from build123d import *

# Parameters (mm, degrees)
SKETCH1_W           = 15
SKETCH1_H           = 20
BOSS_EXTRUDE1_DEPTH = 50
FILLET1_RADIUS      = 10
FILLET1_LENGTH      = 15
SKETCH2_R           = 4
CUT_EXTRUDE1_DEPTH  = 54.150729064
CUT_EXTRUDE2_DEPTH  = 54.150729064
FILLET2_R           = 5
SKETCH4_R           = 3.5
BOSS_EXTRUDE2_DEPTH = 6
DOME1_FACE_RADIUS   = 3.5
DOME1_HEIGHT        = 3
CUT_EXTRUDE3_DEPTH  = 55.371407941


with BuildPart() as part:
    # Sketch1 → Boss-Extrude1 (new body)
    with BuildSketch(Plane(origin=(0, 0, 0), x_dir=(1, 0, 0), z_dir=(0, 1, 0))):
        Rectangle(SKETCH1_W, SKETCH1_H)
    extrude(amount=BOSS_EXTRUDE1_DEPTH)

    # Fillet1: full round fillet: the end face becomes a half cylinder, R = half its width
    fillet1_face = Plane((0, 0, 0), x_dir=(-1, 0, 0), z_dir=(0, -1, 0))  # on the end face: x along it, z out of the body
    fillet1_slab = fillet1_face.offset(-FILLET1_RADIUS / 2) * Box(FILLET1_LENGTH, 2 * FILLET1_RADIUS, FILLET1_RADIUS, mode=Mode.PRIVATE)  # the body's end, R deep
    fillet1_round = Plane((0, 10, 0), x_dir=(0, -1, 0), z_dir=(-1, 0, 0)) * Cylinder(FILLET1_RADIUS, FILLET1_LENGTH, mode=Mode.PRIVATE)  # its axis R under the face
    add(fillet1_slab - fillet1_round, mode=Mode.SUBTRACT)

    # Sketch2 → Cut-Extrude1 (cut, through all)
    with BuildSketch(Plane.ZY.offset(7.5)):
        with Locations((0, 10)):
            Circle(SKETCH2_R)
    extrude(amount=-CUT_EXTRUDE1_DEPTH, mode=Mode.SUBTRACT)

    # Sketch3 → Cut-Extrude2 (cut, through all)
    with BuildSketch(Plane.ZY.offset(7.5)):
        with BuildLine():
            Line((0, 20), (0, 50))
            Line((0, 50), (10, 50))
            Line((10, 50), (10, 10))
            ThreePointArc((10, 10), (7.071067812, 17.071067812), (0, 20))
        make_face()
    extrude(amount=-CUT_EXTRUDE2_DEPTH, mode=Mode.SUBTRACT)

    # Fillet2
    fillet2_edges = [part.edges().sort_by_distance(p)[0] for p in [
        (0, 20, 0),
    ]]
    fillet(fillet2_edges, radius=FILLET2_R)

    # Sketch4 → Boss-Extrude2 (add)
    with BuildSketch(Plane.XY):
        with Locations(Location((0, 25, 0), (0, 0, 194.18798624))):
            Circle(SKETCH4_R)
    extrude(amount=BOSS_EXTRUDE2_DEPTH)

    # Dome1: a dome of height H over a round flat face of radius A is a cap of a sphere of radius (A * A + H * H) / (2 * H)
    dome1_r = (DOME1_FACE_RADIUS * DOME1_FACE_RADIUS + DOME1_HEIGHT * DOME1_HEIGHT) / (2 * DOME1_HEIGHT)
    dome1_base = Plane((0, 25, 6), z_dir=(0, 0, 1))
    with Locations(dome1_base.offset(DOME1_HEIGHT - dome1_r)):
        dome1_ball = Sphere(dome1_r, mode=Mode.PRIVATE)
    add(split(dome1_ball, bisect_by=dome1_base, keep=Keep.TOP, mode=Mode.PRIVATE))

    # Sketch5 → Cut-Extrude3 (cut, through all)
    with BuildSketch(Plane(origin=(0, 0, -10), x_dir=(-1, 0, 0), z_dir=(0, 0, -1))):
        with BuildLine():
            Line((3.05, 50), (3.05, 32.634868852))
            ThreePointArc((3.05, 32.634868852), (0, 29.584868852), (-3.05, 32.634868852))
            Line((-3.05, 32.634868852), (-3.05, 50))
            ThreePointArc((-3.05, 50), (0, 53.05), (3.05, 50))
        make_face()
    extrude(amount=-CUT_EXTRUDE3_DEPTH, mode=Mode.SUBTRACT)


solid = part.part
Can you work these out from the model? Positions are in its coordinate system, mm. A direction names the side the tool comes from. Give positions to 0.01 mm unless a question says otherwise; leave off trailing zeros. Loops run counter-clockwise (first coordinate to the right, second up) from the corner with the lowest first, then second, coordinate; pieces in that order, holes last. Notation, with made-up numbers: M 76,64.5 L 134,64.5 A15 cw 134,79.5 Z; hole C -40,62 d3. An arc over 180 degrees is marked long. One line per item, written item: value. Start each with the question number.
1) If we section it at C-C, the plane z = 2.5: Write out the boundary of the cut face in (x, y).
2) If we section it at B-B, the plane z = -0.5: Write out the boundary of the cut face in (x, y).
3) I'm going to push flat-ended pins straight in: pin 1 (8 mm diameter, centred on x = 1.5, z = 7.5, fed in from +Y); pin 2 (1.5 mm diameter, centred on x = -1, z = -5.5, fed in from +Y); pin 3 (2 mm diameter, centred on x = -2, y = 31, fed in from +Z). Where does each tip first touch, or does it pass through?
4) On a 3-axis mill with a long thin cutter (end or side, diameter ignored), from which of +Z, -Z, +X, -X, +Y, -Y can I reach the whole of each face in a straight line? I mean faces 1 (the face through (5, 50, -5)), 2 (the face through (0.105, 21.291, 0.893)), 3 (the face through (3.05, 41, -5)). Say none if no direction works.
5) Thinking about a two-plate mould opening in Z: for faces 4 (the face through (7.5, 19, -2)), 5 (the face through (-0.105, 13.966, -0.521)), 6 (the face through (-3.4, 36.9, 0)), which applies, +Z half, -Z half, draft (parallel to the pull), parting line (faces both ways), or undercut?
6) If I drill on line 1 (X direction, y = 36, z = -5.5); line 2 (Y direction, x = 0.75, z = 7.25); line 3 (Y direction, x = -2.75, z = 4.5), over which ranges is the centre line in solid material (lowest first)? Write a range as [from, to].
7) If we section it at A-A, the plane x = 6.25: Write out the boundary of the cut face in (y, z).
8) If we section it at D-D, the plane y = 25: Write out the boundary of the cut face in (x, z).
Completed:
1. outline: M -7.5,0.32 L 7.5,0.32 L 7.5,6.88 L -7.5,6.88 Z; M -7.5,13.12 L 7.5,13.12 L 7.5,19.81 L -7.5,19.81 Z; C 0,25 d7
2. outline: M -7.5,0.01 L 7.5,0.01 L 7.5,6.03 L -7.5,6.03 Z; M -7.5,13.97 L 7.5,13.97 L 7.5,50 L 3.05,50 L 3.05,32.63 A3.05 cw -3.05,32.63 L -3.05,50 L -7.5,50 Z
3. pin 1: stops at y = 28.5
3. pin 2: stops at y = 30.14
3. pin 3: stops at z = 0
4. face 1: +Z, -Z, +X, -X, +Y
4. face 2: +Z
4. face 3: +Z, -Z, +Y
5. face 4: draft
5. face 5: undercut
5. face 6: +Z half
6. line 1: x = [-7.5, -3.05], [3.05, 7.5]
6. line 2: y = [3.11, 16.89], [22.04, 27.96]
6. line 3: y = [1.07, 18.93], [22.83, 27.17]
7. outline: M 10,-10 L 50,-10 L 50,0 L 24.14,0 A5 cw 19.43,3.33 A10 ccw long Z; hole C 10,0 d8
8. outline: M -7.5,-10 L 7.5,-10 L 7.5,0 L 3.5,0 L 3.5,6 A3.54 ccw -3.5,6 L -3.5,0 L -7.5,0 Z
